from build123d import *

# Parameters (mm, degrees)
SKETCH1_W = 8
SKETCH1_H = 50


with BuildPart() as part:
    # Sketch1 → Revolve1 (revolve)
    with BuildSketch(Plane(origin=(0, 0, 0), x_dir=(1, 0, 0), z_dir=(0, 1, 0)), mode=Mode.PRIVATE) as revolve1_sk:
        Polygon((-17.5, 94), (0, 94), (0, 112), (-35, 112), (-35, 94), align=None)
        Polygon((-8, 50), (0, 50), (0, 94), (-17.5, 94), (-17.5, 50), align=None)
        with Locations((-4, 25)):
            Rectangle(SKETCH1_W, SKETCH1_H)
    revolve(revolve1_sk.sketch.rotate(Axis((0, 0, 0), (0, 0, -1)), 180), axis=Axis((0, 0, 0), (0, 0, -1)))


solid = part.part
Could you check a few things on this model? Use its own coordinates, in mm. A direction names the side the tool comes from. Give positions to 0.01 mm unless a question says otherwise; leave off trailing zeros. Order: outer loops, then holes, each group sorted by start corner. A loop starts at its lowest first (then second) coordinate and runs counter-clockwise, first axis right, second up. Notation, with made-up numbers: (34, 2.25) -> (87, 2.25) arc R17 ccw to (87, 20.25) -> close; hole circle Ø1 at (83.25, 19). An arc over 180 degrees is marked (long way). Answer in a Markdown table with one row per item. Add a question column.
Item 1: Imagine slicing it at C-C (z = -77.5). List the corners of the cut face in (x, y) for me, and give its area (3 significant figures).
Item 2: Imagine slicing it at B-B (y = 4). List the corners of the cut face in (x, z) for me.
Item 3: Imagine slicing it at A-A (x = 0). List the corners of the cut face in (y, z) for me.
Item 4: Please list where these lines run through material, in increasing order: probe 1 along Z at (x, y) = (-21, 13); probe 2 along Z at (x, y) = (11.5, 9.5); probe 3 along X at (y, z) = (-1, -106).
Item 5: I'm going to push flat-ended pins straight in: P1, Ø5, axis at y = -12.5, z = -92, coming from the +X side; P2, Ø6, axis at x = 10.5, z = -50.5, coming from the +Y side; P3, Ø3, axis at x = 5.5, y = 21, coming from the +Z side. Where does each tip first touch, or does it pass through?
Item 6: Imagine slicing it at D-D (x = -13). List the corners of the cut face in (y, z) for me, and give its area (3 significant figures).
Item 7: For faces 1 (the cylindrical face through (-7.587, 34.168, -102.874)), 2 (the flat face through (4, 8, -50)), which set-ups out of +Z, -Z, +X, -X, +Y, -Y let a thin tool reach every point of the face, with its end or its side?
Result:
| question | item | result |
|---|---|---|
| 1 | outline | circle Ø35 at (0, 0) |
| 1 | area | 962 mm2 |
| 2 | outline | (-34.77, -112) -> (34.77, -112) -> (34.77, -94) -> (17.04, -94) -> (17.04, -50) -> (6.93, -50) -> (6.93, 0) -> (-6.93, 0) -> (-6.93, -50) -> (-17.04, -50) -> (-17.04, -94) -> (-34.77, -94) -> close |
| 3 | outline | (-35, -112) -> (35, -112) -> (35, -94) -> (17.5, -94) -> (17.5, -50) -> (8, -50) -> (8, 0) -> (-8, 0) -> (-8, -50) -> (-17.5, -50) -> (-17.5, -94) -> (-35, -94) -> close |
| 4 | probe 1 | -112 to -94 |
| 4 | probe 2 | -112 to -50 |
| 4 | probe 3 | -34.99 to 34.99 |
| 5 | P1 | x = 33.23 |
| 5 | P2 | y = 15.81 |
| 5 | P3 | z = -94 |
| 6 | outline | (-32.5, -112) -> (32.5, -112) -> (32.5, -94) -> (11.72, -94) -> (11.72, -50) -> (-11.72, -50) -> (-11.72, -94) -> (-32.5, -94) -> close |
| 6 | area | 2,200 mm2 |
| 7 | face 1 | +Z, -Z |
| 7 | face 2 | +Z |
